from build123d import *

# Parameters (mm, degrees)
SKETCH_1_W          = 215
SKETCH_1_H          = 250
EXTRUDE_1_DEPTH     = 7
SKETCH_2_W          = 57
SKETCH_2_H          = 250
CUT_EXTRUDE_1_DEPTH = 1.5
CHAMFER_1_SIZE      = 2


with BuildPart() as part:
    # 草图1 → 凸台-拉伸1 (new, symmetric)
    with BuildSketch(Plane(origin=(0, 0, 0), x_dir=(1, 0, 0), z_dir=(0, 1, 0))):
        Rectangle(SKETCH_1_W, SKETCH_1_H)
    extrude(amount=EXTRUDE_1_DEPTH, both=True)

    # 草图2 → 切除-拉伸1 (cut)
    with BuildSketch(Plane.XZ.offset(7)):
        with Locations((79, 0)):
            Rectangle(SKETCH_2_W, SKETCH_2_H)
        with Locations((-79, 0)):
            Rectangle(SKETCH_2_W, SKETCH_2_H)
    extrude(amount=-CUT_EXTRUDE_1_DEPTH, mode=Mode.SUBTRACT)

    # 倒角1
    chamfer_1_edges = [part.edges().sort_by_distance(p)[0] for p in [
        (107.5, 0.75, 125),
        (-107.5, 0.75, 125),
        (-107.5, 0.75, -125),
        (107.5, 0.75, -125),
    ]]
    chamfer(chamfer_1_edges, length=CHAMFER_1_SIZE)


solid = part.part
Here's how the part is built. I have some questions about the finished solid (model axes, mm). A direction names the side the tool comes from. Coordinates: 2 decimals unless noted, no trailing zeros. Order: outer loops, then holes, each group sorted by start corner. A loop starts at its lowest first (then second) coordinate and runs counter-clockwise, first axis right, second up. Notation, with made-up numbers: M 12.5,22 L 20.5,22 A17 ccw 20.5,36 Z; hole C 23,45 d3. An arc over 180 degrees is marked long. Answer as CSV lines item,"result".
Item 1: For pin 1 (0.8 mm diameter, centred on y = -6, z = 1.5, fed in from -X), with a flat end and sliding along its axis, tell me the tip position at first contact or that it passes through.
Results found:
pin 1,"x = -50.5"
Item 2: Imagine slicing it at A-A on z = 58. Write out the boundary of the cut face in (x, y).
Results found:
outline,"M -107.5,-5.5 L -50.5,-5.5 L -50.5,-7 L 50.5,-7 L 50.5,-5.5 L 107.5,-5.5 L 107.5,7 L -107.5,7 Z"
Item 3: Imagine slicing it at B-B on x = 65. Write out the boundary of the cut face in (y, z).
Results found:
outline,"M -5.5,-125 L 7,-125 L 7,125 L -5.5,125 Z"
Item 4: If I drill on line 1 (Y direction, x = -69.5, z = 89); line 2 (X direction, y = -5.75, z = -88), over which ranges is the centre line in solid material (lowest first)?
Results found:
line 1,"-5.5 to 7"
line 2,"-50.5 to 50.5"
Item 5: On a 3-axis mill with a long thin cutter (end or side, diameter ignored), from which of +Z, -Z, +X, -X, +Y, -Y can I reach the whole of each face in a straight line? I mean faces 1 (the face through (79, -5.5, 2)), 2 (the face through (-107.5, 1, 2)), 3 (the face through (-79, -5.5, 2)). Say none if no direction works.
Results found:
face 1,"+Z, -Z, +X, -Y"
face 2,"+Z, -Z, -X, +Y, -Y"
face 3,"+Z, -Z, -X, -Y"
